The model under review builds one solid part; all positions refer to its coordinate system, in mm. Face numbers are marked on the shaded views. A direction names the side the tool comes from. Round coordinates to 2 decimals unless told otherwise and drop trailing zeros. Order: outer loops, then holes, each group sorted by start corner. A loop starts at its lowest first (then second) coordinate and runs counter-clockwise, first axis right, second up. Notation, with made-up numbers: (74.5, 12) - (93.5, 12) arc R37 ccw to (93.5, 50) - close; hole circle Ø6 at (70, -20). An arc over 180 degrees is marked (long way). One line per question, with ' | ' between items. Start each with the question number.
Item 1: Insertion check: pin 1 Ø0.8 at (x, y) = (62, 1) entering from +Z; pin 2 Ø3 at (x, y) = (-30, 27) entering from +Z; pin 3 Ø7.5 at (x, z) = (29.5, -11.5) entering from -Y; pin 4 Ø1 at (y, z) = (27.5, 5.5) entering from -X. Each pin has a flat end and moves straight along its axis. Give the tip position at first contact, or say it passes through.
Item 2: Add section B-B on y = 27. State the section outline as (x, z) points.
Item 3: Tool access review of the marked faces 4, 5, 6 and 7: name each direction out of +Z, -Z, +X, -X, +Y, -Y from which nothing blocks a thin tool from reaching the whole face with its end or side.
Item 4: Add section D-D on z = 9. State the section outline as (x, y) points.
Item 5: For L1, parallel to Y at x = -30, z = -8.5; L2, parallel to X at y = 3, z = -3; L3, parallel to X at y = 2.5, z = 5, list the stretches that pass through material, from the lowest coordinate up. Write a range as [from, to].
Item 6: Add section A-A on z = 0. State the section outline as (x, y) points, and give its area (3 significant figures).
Item 7: Add section C-C on z = -10. State the section outline as (x, y) points.
Item 8: Draft analysis for pull direction X (two halves, no side actions). For the marked faces 1, 2 and 3, state which applies: +X half, -X half, draft (parallel to the pull), parting line (faces both ways), or undercut.
from build123d import *

# Parameters (mm, degrees)
EXTRUDE_1_DEPTH        = 15
SKETCH_2_W             = 7.5
SKETCH_2_H             = 3
CUT_EXTRUDE_1_DEPTH    = 155.757875405
SKETCH_3_W             = 100
SKETCH_3_H             = 20
CUT_EXTRUDE_2_DEPTH    = 85.113019206
CUT_EXTRUDE_3_DEPTH    = 30
HOLE_WIZARD_M6_1_D     = 5
PATTERN_LINEAR_1_COUNT = 2
PATTERN_LINEAR_1_PITCH = 10
CHAMFER_1_SIZE         = 0.5
SKETCH_7_R             = 1
CUT_EXTRUDE_4_DEPTH    = 85.113019206


with BuildPart() as part:
    # 草图1 → 凸台-拉伸1 (new, symmetric)
    with BuildSketch(Plane.XY):
        Polygon((-75, 0), (-75, 15), (-55, 15), (-55, 35), (55, 35), (55, 15), (75, 15), (75, 0), align=None)
    extrude(amount=EXTRUDE_1_DEPTH, both=True)

    # 草图2 → 切除-拉伸1 (cut, through all)
    with BuildSketch(Plane.ZY.offset(75)):
        with Locations((-11.25, 1.5)):
            Rectangle(SKETCH_2_W, SKETCH_2_H)
        with Locations((11.25, 1.5)):
            Rectangle(SKETCH_2_W, SKETCH_2_H)
    extrude(amount=-CUT_EXTRUDE_1_DEPTH, mode=Mode.SUBTRACT)

    # 草图3 → 切除-拉伸2 (cut, through all)
    with BuildSketch(Plane(origin=(0, 35, 0), x_dir=(1, 0, 0), z_dir=(0, 1, 0))):
        with Locations((0, -5)):
            Rectangle(SKETCH_3_W, SKETCH_3_H)
    extrude(amount=-CUT_EXTRUDE_2_DEPTH, mode=Mode.SUBTRACT)

    # 草图4 → 切除-拉伸3 (cut)
    with BuildSketch(Plane(origin=(0, 15, 0), x_dir=(1, 0, 0), z_dir=(0, 1, 0))):
        with BuildLine():
            Line((61, 3.25), (69, 3.25))
            ThreePointArc((69, 3.25), (72.25, 0), (69, -3.25))
            Line((69, -3.25), (61, -3.25))
            ThreePointArc((61, -3.25), (57.75, 0), (61, 3.25))
        make_face()
        with BuildLine():
            Line((-61, 3.25), (-69, 3.25))
            ThreePointArc((-69, 3.25), (-72.25, 0), (-69, -3.25))
            Line((-69, -3.25), (-61, -3.25))
            ThreePointArc((-61, -3.25), (-57.75, 0), (-61, 3.25))
        make_face()
    extrude(amount=-CUT_EXTRUDE_3_DEPTH, mode=Mode.SUBTRACT)

    # M6 螺纹孔1 (through all)
    with Locations(Plane.XY.offset(-5)):
        with Locations((-30, 17), (30, 17)):
            hole_wizard_m6_1 = Hole(HOLE_WIZARD_M6_1_D / 2)

    # 阵列(线性)1: M6 螺纹孔1 ×2
    with Locations(*[(0, i * PATTERN_LINEAR_1_PITCH, 0) for i in range(1, PATTERN_LINEAR_1_COUNT)]):
        add(hole_wizard_m6_1, mode=Mode.SUBTRACT)

    # 倒角1
    chamfer_1_edges = [part.edges().sort_by_distance(p)[0] for p in [
        (55, 25, -15),
        (65, 15, -15),
        (32.5, 17, -15),
        (-27.5, 17, -15),
        (32.5, 27, -15),
        (65, 15, 15),
        (-27.5, 27, -15),
        (-75, 15, 0),
        (-55, 35, 0),
        (55, 35, 0),
        (75, 15, 0),
        (55, 25, 15),
        (52.5, 35, 15),
        (75, 9, -15),
        (-55, 25, 15),
        (75, 9, 15),
        (-75, 0, 0),
        (-65, 15, 15),
        (75, 0, 0),
        (75, 3, -11.25),
        (-75, 9, 15),
        (0, 3, -15),
        (75, 1.5, -7.5),
        (0, 0, -7.5),
        (-75, 1.5, -7.5),
        (-75, 3, -11.25),
        (75, 1.5, 7.5),
        (62.5, 0, 7.5),
        (75, 3, 11.25),
        (62.5, 3, 15),
        (-75, 3, 11.25),
        (-75, 1.5, 7.5),
        (-62.5, 3, 15),
        (-62.5, 0, 7.5),
        (-52.5, 35, 15),
        (-50, 19, 15),
        (50, 19, 15),
        (-75, 9, -15),
        (-65, 15, -15),
        (-55, 25, -15),
        (0, 35, -15),
    ]]
    chamfer(chamfer_1_edges, length=CHAMFER_1_SIZE)

    # 草图7 → 切除-拉伸4 (cut, through all)
    with BuildSketch(Plane(origin=(0, 35, 0), x_dir=(1, 0, 0), z_dir=(0, 1, 0))):
        with Locations((-49, 5)):
            Circle(SKETCH_7_R)
        with Locations((49, 5)):
            Circle(SKETCH_7_R)
    extrude(amount=-CUT_EXTRUDE_4_DEPTH, mode=Mode.SUBTRACT)


solid = part.part
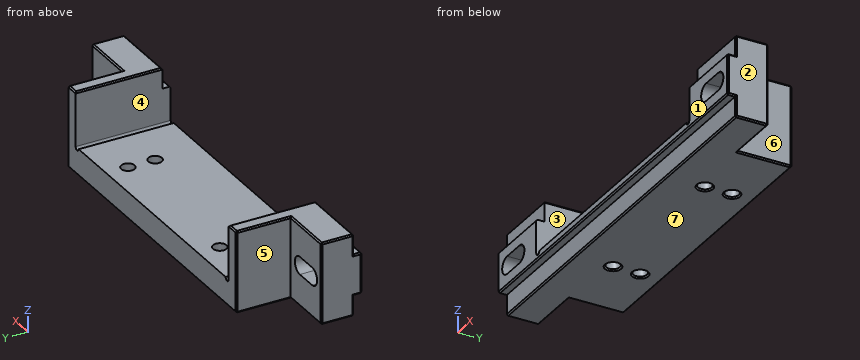
Determined:
1) pin 1: z = 7.5 | pin 2: through | pin 3: y = 3 | pin 4: x = -55
2) outline: (-55, -14.5) - (-54.5, -15) - (-33, -15) - (-32.5, -14.5) - (-32.5, -5) - (-48, -5) arc R1 cw to (-50, -5) - (-50, 14.5) - (-50.5, 15) - (-54.5, 15) - (-55, 14.5) - close; (-27.5, -14.5) - (-27, -15) - (27, -15) - (27.5, -14.5) - (27.5, -5) - (-27.5, -5) - close; (32.5, -14.5) - (33, -15) - (54.5, -15) - (55, -14.5) - (55, 14.5) - (54.5, 15) - (50.5, 15) - (50, 14.5) - (50, -5) arc R1 cw to (48, -5) - (32.5, -5) - close
3) face 4: +Z, +Y, -Y | face 5: +Z, -Z, -X, +Y | face 6: +Z, -Z, +X, +Y | face 7: -Z, +X, -X, +Y, -Y
4) outline: (-75, 3.5) - (-74.5, 3) - (-50, 3) - (-50, 35) - (-54.5, 35) - (-55, 34.5) - (-55, 15) - (-74.5, 15) - (-75, 14.5) - close; (50, 3) - (74.5, 3) - (75, 3.5) - (75, 14.5) - (74.5, 15) - (55, 15) - (55, 34.5) - (54.5, 35) - (50, 35) - close
5) L1: [3, 14.5], [19.5, 24.5], [29.5, 35] | L2: [-75, -70.25], [-59.75, -50], [50, 59.75], [70.25, 75] | L3: [-75, -50], [50, 75]
6) outline: (-75, 0.5) - (-74.5, 0) - (-72.25, 0) - (-72.25, 15) - (-74.5, 15) - (-75, 14.5) - close; (-57.75, 0) - (-50, 0) - (-50, 35) - (-54.5, 35) - (-55, 34.5) - (-55, 15) - (-57.75, 15) - close; (50, 0) - (57.75, 0) - (57.75, 15) - (55, 15) - (55, 34.5) - (54.5, 35) - (50, 35) - close; (72.25, 0) - (74.5, 0) - (75, 0.5) - (75, 14.5) - (74.5, 15) - (72.25, 15) - close | area: 514 mm2
7) outline: (-75, 3.5) - (-74.5, 3) - (74.5, 3) - (75, 3.5) - (75, 14.5) - (74.5, 15) - (55, 15) - (55, 34.5) - (54.5, 35) - (-54.5, 35) - (-55, 34.5) - (-55, 15) - (-74.5, 15) - (-75, 14.5) - close; hole circle Ø5 at (-30, 17); hole circle Ø5 at (-30, 27); hole circle Ø5 at (30, 17); hole circle Ø5 at (30, 27)
8) face 1: draft | face 2: +X half | face 3: undercut
